Verification items for this drawing (mm, ordinates from the low corner). Give positions to 0.01 mm unless a question says otherwise; leave off trailing zeros. Write each loop counter-clockwise with the first axis right and the second up, starting at its lowest first coordinate (ties: lowest second). Pieces come first, ordered by that corner, then holes. Notation, with made-up numbers: M 72,5 L 84,5 A25 ccw 84,43 Z; hole C 3.5,4.25 d7. An arc over 180 degrees is marked long. Use one line per item in the form item = value. Start each with the question number.
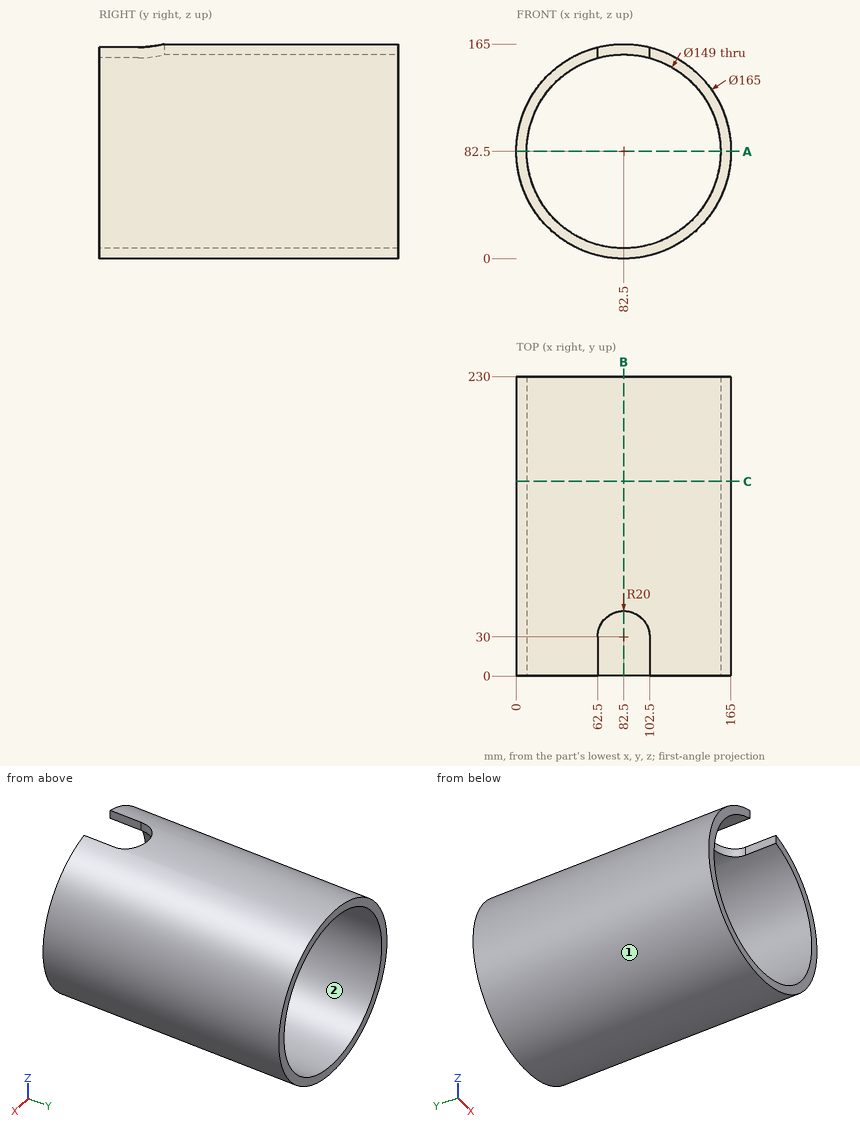
(1) Sectioned sample at A-A, the plane z = 82.5. Record the boundary of the cut face in (x, y), plus the area to 3 significant figures.
(2) Thickness scan on probe 1 along Z at (x, y) = (82, 105); probe 2 along Z at (x, y) = (102.5, 90.5). Record the ranges inside material, lowest first. Write a range as [from, to].
(3) Draft check along X on the marked faces 1 and 2. Enter one of: released by +X, released by -X, zero draft, split by the parting line, or undercut.
(4) Sectioned sample at B-B, the plane x = 82.5. Record the boundary of the cut face in (y, z), plus the area to 3 significant figures.
(5) Sectioned sample at C-C, the plane y = 149.5. Record the boundary of the cut face in (x, z), plus the area to 3 significant figures.
(6) Depth check by flat-ended pin: pin 1 (8 mm diameter, centred on y = 67.5, z = 54, fed in from -X); pin 2 (6 mm diameter, centred on x = 111.5, y = 37, fed in from -Z); pin 3 (6 mm diameter, centred on x = 122, y = 198.5, fed in from +Z). Enter the tip coordinate at first touch or a pass-through.
Numbers:
q1.outline = M 0,0 L 8,0 L 8,230 L 0,230 Z; M 157,0 L 165,0 L 165,230 L 157,230 Z
q1.area = 3,680 mm2
q2.probe_1 = [0, 8], [157, 165]
q2.probe_2 = [2.46, 10.73], [154.27, 162.54]
q3.face_1 = split by the parting line
q3.face_2 = undercut
q4.outline = M 0,0 L 230,0 L 230,8 L 0,8 Z; M 50,157 L 230,157 L 230,165 L 50,165 Z
q4.area = 3,280 mm2
q5.outline = C 82.5,82.5 d165; hole C 82.5,82.5 d149
q5.area = 3,950 mm2
q6.pin_1 = 3.72
q6.pin_2 = 4.2
q6.pin_3 = 156.49
